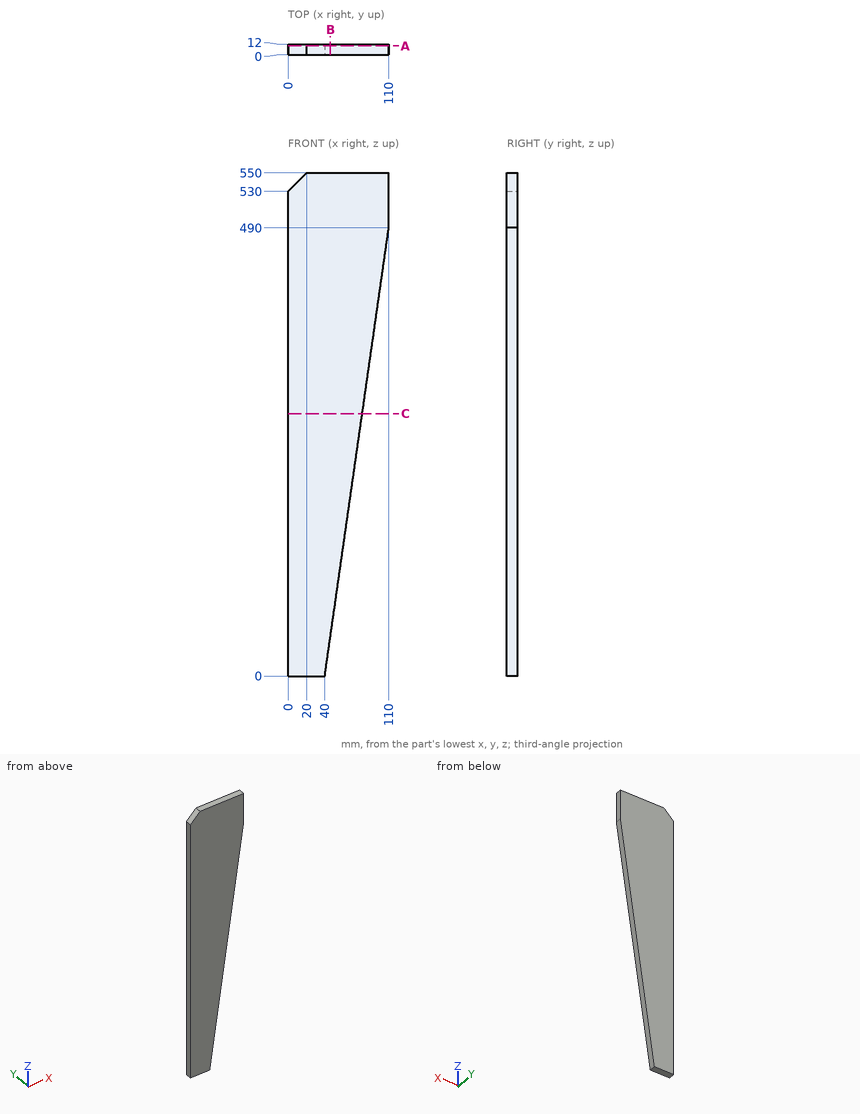
Geometry: see drawing. Coordinates: mm, zero at the bounding-box minimum. Coordinates: 2 decimals unless noted, no trailing zeros. Order: outer loops, then holes, each group sorted by start corner. A loop starts at its lowest first (then second) coordinate and runs counter-clockwise, first axis right, second up. Notation, with made-up numbers: M 22.5,54.5 L 31.5,54.5 A30 ccw 31.5,89.5 Z; hole C 83.25,76.5 d6. An arc over 180 degrees is marked long. Answer in a Markdown table with one row per item. Add a question column.
Q1. Contact query for a flat-ended pin moving along its axis: P1, Ø6, axis at y = 5, z = 391, coming from the +X side. Output: stop coordinate, or through.
Q2. Line query: L1, parallel to X at y = 11.25, z = 91; L2, parallel to X at y = 5, z = 75.5; L3, parallel to Z at x = 17, y = 3. Output: solid intervals per line, ascending.
Q3. Section query C-C on z = 287. Return the cut outline in (x, y).
Q4. Section query A-A on y = 10. Return the cut outline in (x, z).
Q5. Section query B-B on x = 46. Return the cut outline in (y, z), and give its area (3 significant figures).
Completed:
| question | item | result |
|---|---|---|
| 1 | P1 | stops at x = 96.29 |
| 2 | L1 | x = 0 to 53 |
| 2 | L2 | x = 0 to 50.79 |
| 2 | L3 | z = 0 to 547 |
| 3 | outline | M 0,0 L 81,0 L 81,12 L 0,12 Z |
| 4 | outline | M 0,0 L 40,0 L 110,490 L 110,550 L 20,550 L 0,530 Z |
| 5 | outline | M 0,42 L 12,42 L 12,550 L 0,550 Z |
| 5 | area | 6,100 mm2 |
